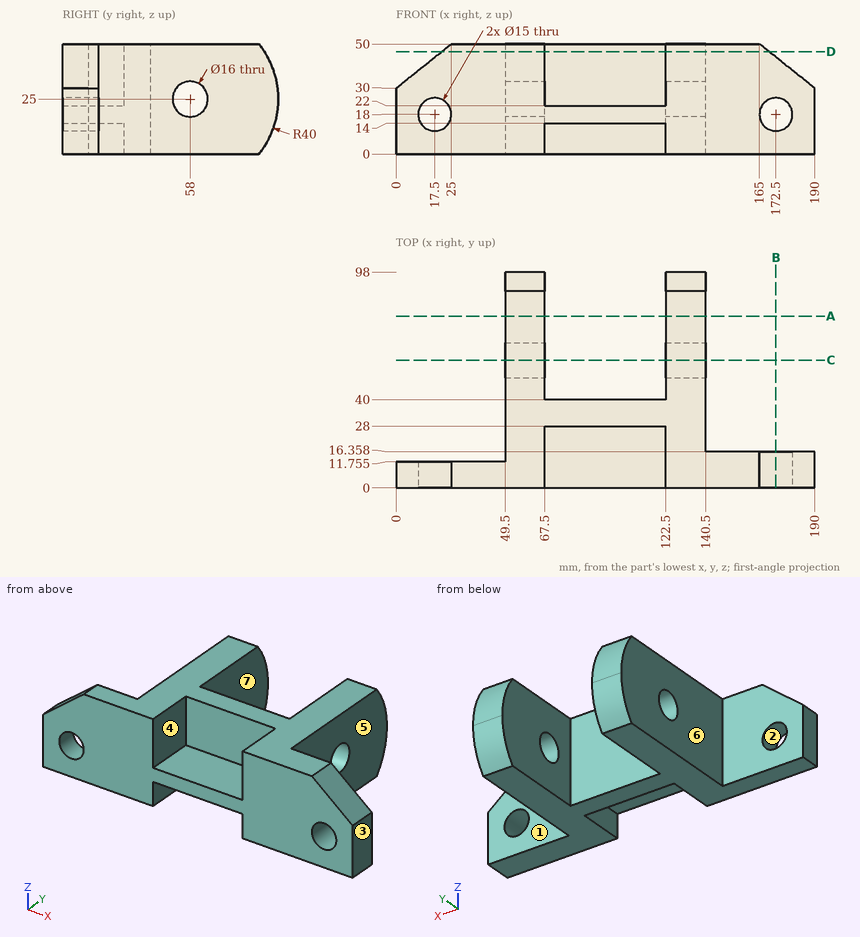
Geometry check sheet. Reference: drawing and pictorial views, mm from the part's lowest x, y, z. A direction names the side the tool comes from. Round coordinates to 2 decimals unless told otherwise and drop trailing zeros. Order: outer loops, then holes, each group sorted by start corner. A loop starts at its lowest first (then second) coordinate and runs counter-clockwise, first axis right, second up. Notation, with made-up numbers: M -18.5,-8.5 L 17.5,-8.5 A30 ccw 17.5,24.5 Z; hole C 60.5,18 d5. An arc over 180 degrees is marked long. Answer in a Markdown table with one row per item.
(1) Sectioned sample at B-B, the plane x = 172.5. Record the cut outline in (y, z).
Responses:
| item | result |
|---|---|
| outline | M 0,0 L 16.36,0 L 16.36,10.5 L 0,10.5 Z; M 0,25.5 L 16.36,25.5 L 16.36,44 L 0,44 Z |
(2) Go/stop test with flat-tipped pins: P1, Ø25, axis at x = 99.5, z = 33, coming from the +Y side; P2, Ø12, axis at x = 20, z = 16, coming from the -Y side; P3, Ø15, axis at x = 22.5, z = 30, coming from the +Y side (1 decimal); P4, Ø8.5, axis at y = 10.5, z = 38.5, coming from the -X side. Record where each tip stops, or that it passes through.
Responses:
| item | result |
|---|---|
| P1 | stops at y = 40 |
| P2 | stops at y = 0 |
| P3 | stops at y = 11.8 |
| P4 | stops at x = 5.31 |
(3) Draft check along X on the marked faces 1, 2 and 3. Enter one of: released by +X, released by -X, zero draft, split by the parting line, or undercut.
Responses:
| item | result |
|---|---|
| face 1 | zero draft |
| face 2 | undercut |
| face 3 | released by +X |
(4) Scan lines: probe 1 along X at (y, z) = (3.5, 18); probe 2 along X at (y, z) = (50.5, 30); probe 3 along Y at (x, z) = (94.5, 43). Record each from-to range of solid material in increasing order. Write a range as from..to.
Responses:
| item | result |
|---|---|
| probe 1 | x = 0..10, 25..165, 180..190 |
| probe 2 | x = 49.5..67.5, 122.5..140.5 |
| probe 3 | y = 28..40 |
(5) Sectioned sample at C-C, the plane y = 58. Record the cut outline in (x, z).
Responses:
| item | result |
|---|---|
| outline | M 49.5,0 L 67.5,0 L 67.5,17 L 49.5,17 Z; M 49.5,33 L 67.5,33 L 67.5,50 L 49.5,50 Z; M 122.5,0 L 140.5,0 L 140.5,17 L 122.5,17 Z; M 122.5,33 L 140.5,33 L 140.5,50 L 122.5,50 Z |
(6) Sectioned sample at D-D, the plane z = 46.5. Record the cut outline in (x, y) (1 decimal).
Responses:
| item | result |
|---|---|
| outline | M 20.6,0 L 67.5,0 L 67.5,28 L 122.5,28 L 122.5,0 L 169.4,0 L 169.4,16.4 L 140.5,16.4 L 140.5,91.7 L 122.5,91.7 L 122.5,40 L 67.5,40 L 67.5,91.7 L 49.5,91.7 L 49.5,11.8 L 20.6,11.8 Z |
(7) Sectioned sample at A-A, the plane y = 78. Record the cut outline in (x, z), and give its area (3 significant figures).
Responses:
| item | result |
|---|---|
| outline | M 49.5,0 L 67.5,0 L 67.5,50 L 49.5,50 Z; M 122.5,0 L 140.5,0 L 140.5,50 L 122.5,50 Z |
| area | 1,800 mm² |
(8) Tool access check on the marked faces 4, 5, 6 and 7. Record the directions out of +Z, -Z, +X, -X, +Y, -Y that give a thin tool (end or side, any length) a straight path to the whole face; none if there is none.
Responses:
| item | result |
|---|---|
| face 4 | +Z, -Y |
| face 5 | +Z, -Z, +X, +Y |
| face 6 | +Z, -Z, -X, +Y |
| face 7 | +Z, -Z, +Y |
